Check sheet for the modelled part. Datum: model origin and axes. Units: mm. A direction names the side the tool comes from. Coordinates: 2 decimals unless noted, no trailing zeros. Write each loop counter-clockwise with the first axis right and the second up, starting at its lowest first coordinate (ties: lowest second). Pieces come first, ordered by that corner, then holes. Notation, with made-up numbers: (34, 85) -> (44, 85) arc R8 ccw to (44, 95) -> close; hole circle Ø4 at (-37.75, 10.5). An arc over 180 degrees is marked (long way). Put each result on its own line as item: value.
```python
from build123d import *

# Parameters (mm, degrees)
SKETCH1_R           = 5
BOSS_EXTRUDE1_DEPTH = 110
CUT_EXTRUDE1_DEPTH  = 111.227038425
CUT_EXTRUDE2_START  = -10
CUT_EXTRUDE2_DEPTH  = 10
M4_TAPPED_HOLE2_D   = 3.3


with BuildPart() as part:
    # Sketch1 → Boss-Extrude1 (new body)
    with BuildSketch(Plane(origin=(0, 0, 0), x_dir=(1, 0, 0), z_dir=(0, 1, 0))):
        with Locations(Location((0, 0, 0), (0, 0, 270))):
            Circle(SKETCH1_R)
    extrude(amount=BOSS_EXTRUDE1_DEPTH)

    # Sketch2 → Cut-Extrude1 (cut, through all)
    with BuildSketch(Plane(origin=(0, 110, 0), x_dir=(1, 0, 0), z_dir=(0, 1, 0))):
        with BuildLine():
            Line((-4, -3), (4, -3))
            ThreePointArc((4, -3), (0, -5), (-4, -3))
        make_face()
    extrude(amount=-CUT_EXTRUDE1_DEPTH, mode=Mode.SUBTRACT)

    # Sketch3 → Cut-Extrude2 (cut)
    with BuildSketch(Plane(origin=(0, 110, 0), x_dir=(1, 0, 0), z_dir=(0, 1, 0)).offset(CUT_EXTRUDE2_START)):
        with BuildLine():
            Line((-4.582575695, 2), (4.582575695, 2))
            ThreePointArc((4.582575695, 2), (0, 5), (-4.582575695, 2))
        make_face()
    cut_extrude2 = extrude(amount=CUT_EXTRUDE2_DEPTH, mode=Mode.SUBTRACT)

    # Mirror1: Cut-Extrude2 across plane
    add(cut_extrude2.mirror(Plane.ZX.offset(55)), mode=Mode.SUBTRACT)

    # M4 Tapped Hole2 (through all)
    with Locations(Plane(origin=(0, 0, -2), x_dir=(-1, 0, 0), z_dir=(0, 0, -1))):
        with Locations((0, 104), (0, 6)):
            Hole(M4_TAPPED_HOLE2_D / 2)


solid = part.part
```
Q1. Cross-section at C-C (z = 0.5). Record the cut outline in (x, y), plus the area to 3 significant figures.
Recorded:
outline: (-4.97, 0) -> (4.97, 0) -> (4.97, 110) -> (-4.97, 110) -> close; hole circle Ø3.3 at (0, 6); hole circle Ø3.3 at (0, 104)
area: 1,080 mm2
Q2. Depth check by flat-ended pin: P1, Ø4.5, axis at x = 0, y = 104, coming from the -Z side; P2, Ø1.5, axis at x = -1, z = -4, coming from the +Y side. Enter the tip coordinate at first touch or a pass-through.
Recorded:
P1: stops at z = -2
P2: stops at y = 100
Q3. Mould release check, pull along X, two halves, no side actions. Record for faces 1 (the flat face through (0, 56, 3)), 2 (the cylindrical face through (0, 54, -5)), 3 (the cylindrical face through (-0.4, 4.4, 0.5)): released by +X, released by -X, zero draft, split by the parting line, or undercut.
Recorded:
face 1: zero draft
face 2: split by the parting line
face 3: undercut
Q4. Material ranges on line 1 along Y through (x, z) = (0, -0.2); line 2 along X through (y, z) = (104, -0.4); line 3 along Y through (x, z) = (1.5, 1.25), recorded low to high.
Recorded:
line 1: y = 0 to 4.35, 7.65 to 102.35, 105.65 to 110
line 2: x = -4.98 to -1.65, 1.65 to 4.98
line 3: y = 0 to 5.31, 6.69 to 103.31, 104.69 to 110
Q5. Tool access check on faces 4 (the flat face through (0, 0, 0)), 5 (the flat face through (0, 10, -3)), 6 (the flat face through (0, 100, -3)). Record the directions out of +Z, -Z, +X, -X, +Y, -Y that give a thin tool (end or side, any length) a straight path to the whole face; none if there is none.
Recorded:
face 4: +Z, -Z, +X, -X, -Y
face 5: -Z, +X, -X, -Y
face 6: -Z, +X, -X, +Y
Q6. Cross-section at B-B (y = 6). Record the cut outline in (x, z).
Recorded:
outline: (-4.58, -2) -> (-1.65, -2) -> (-1.65, 3) -> (-4, 3) arc R5 ccw to start; (1.65, -2) -> (4.58, -2) arc R5 ccw to (4, 3) -> (1.65, 3) -> close
Q7. Cross-section at A-A (x = 0). Record the cut outline in (y, z), plus the area to 3 significant figures.
Recorded:
outline: (0, -2) -> (4.35, -2) -> (4.35, 3) -> (0, 3) -> close; (7.65, -2) -> (10, -2) -> (10, -5) -> (100, -5) -> (100, -2) -> (102.35, -2) -> (102.35, 3) -> (7.65, 3) -> close; (105.65, -2) -> (110, -2) -> (110, 3) -> (105.65, 3) -> close
area: 787 mm2
Q8. Cross-section at D-D (y = 45). Record the cut outline in (x, z), plus the area to 3 significant figures.
Recorded:
outline: (-4, 3) arc R5 ccw (long way) to (4, 3) -> close
area: 67.4 mm2
